```python
from build123d import *

# Parameters (mm, degrees)
SKETCH_1_R          = 21
SKETCH_1_R_2        = 7.5
EXTRUDE_1_DEPTH     = 13
EXTRUDE_2_DEPTH     = 6.5
FILLET_1_R          = 4
FILLET_2_R          = 2
SKETCH_3_R          = 3.5
CUT_EXTRUDE_1_DEPTH = 6.5
SKETCH_4_R          = 18
CUT_EXTRUDE_2_DEPTH = 2


with BuildPart() as part:
    # 草图1 → 凸台-拉伸1 (new body)
    with BuildSketch(Plane(origin=(0, 0, 0), x_dir=(1, 0, 0), z_dir=(0, 1, 0))):
        with Locations(Location((0, 0, 0), (0, 0, 90))):
            Circle(SKETCH_1_R)
        with Locations(Location((0, 0, 0), (0, 0, 90))):
            Circle(SKETCH_1_R_2, mode=Mode.SUBTRACT)
    extrude(amount=EXTRUDE_1_DEPTH)

    # 草图2 → 凸台-拉伸2 (add)
    with BuildSketch(Plane.XZ):
        with BuildLine():
            Line((32.727876998, 4.229192264), (19.975971523, 6.477697255))
            ThreePointArc((19.975971523, 6.477697255), (21, 0), (19.975971523, -6.477697255))
            Line((19.975971523, -6.477697255), (32.727876998, -4.229192264))
            ThreePointArc((32.727876998, -4.229192264), (33, 0), (32.727876998, 4.229192264))
        make_face()
        with BuildLine():
            Line((-32.727876998, -4.229192264), (-19.975971523, -6.477697255))
            ThreePointArc((-19.975971523, -6.477697255), (-21, 0), (-19.975971523, 6.477697255))
            Line((-19.975971523, 6.477697255), (-32.727876998, 4.229192264))
            ThreePointArc((-32.727876998, 4.229192264), (-33, 0), (-32.727876998, -4.229192264))
        make_face()
    extrude(amount=-EXTRUDE_2_DEPTH)

    # 圆角1
    fillet_1_edges = [part.edges().sort_by_distance(p)[0] for p in [
        (19.975971523, 3.25, -6.477697255),
        (19.975971523, 3.25, 6.477697255),
        (-19.975971523, 3.25, 6.477697255),
        (-19.975971523, 3.25, -6.477697255),
    ]]
    fillet(fillet_1_edges, radius=FILLET_1_R)

    # 圆角2
    fillet_2_edges = [part.edges().sort_by_distance(p)[0] for p in [
        (32.727876998, 3.25, 4.229192264),
        (32.727876998, 3.25, -4.229192264),
        (-32.727876998, 3.25, -4.229192264),
        (-32.727876998, 3.25, 4.229192264),
    ]]
    fillet(fillet_2_edges, radius=FILLET_2_R)

    # 草图3 → 切除-拉伸1 (cut)
    with BuildSketch(Plane(origin=(0, 6.5, 0), x_dir=(1, 0, 0), z_dir=(0, 1, 0))):
        with Locations(Location((-26.5, 0, 0), (0, 0, 270))):
            Circle(SKETCH_3_R)
        with Locations(Location((26.5, 0, 0), (0, 0, 270))):
            Circle(SKETCH_3_R)
    extrude(amount=-CUT_EXTRUDE_1_DEPTH, mode=Mode.SUBTRACT)

    # 草图4 → 切除-拉伸2 (cut)
    with BuildSketch(Plane.XZ):
        with Locations(Location((0, 0, 0), (0, 0, 270))):
            Circle(SKETCH_4_R)
    extrude(amount=-CUT_EXTRUDE_2_DEPTH, mode=Mode.SUBTRACT)


solid = part.part
```
Check sheet for the modelled part. Datum: model origin and axes. Units: mm. Give positions to 0.01 mm unless a question says otherwise; leave off trailing zeros. Loops run counter-clockwise (first coordinate to the right, second up) from the corner with the lowest first, then second, coordinate; pieces in that order, holes last. Notation, with made-up numbers: M 49,-24 L 61,-24 A5 cw 61,-17 Z; hole C 57.5,-14 d4. An arc over 180 degrees is marked long. Answer as CSV lines item,"result".
Item 1: Sectioned sample at D-D, the plane z = -10.5. Enter the section's corners in (x, y).
Reply:
outline,"M -18.19,0 L -14.62,0 L -14.62,2 L 14.62,2 L 14.62,0 L 18.19,0 L 18.19,13 L -18.19,13 Z"
Item 2: Sectioned sample at A-A, the plane x = 0. Enter the section's corners in (y, z), then the cut area to 3 significant figures.
Reply:
outline,"M 0,-21 L 13,-21 L 13,-7.5 L 2,-7.5 L 2,-18 L 0,-18 Z; M 0,18 L 2,18 L 2,7.5 L 13,7.5 L 13,21 L 0,21 Z"
area,"309 mm^2"
Item 3: Draft check along Z on faces 1 (the face through (-0.33, 7.423, 7.493)), 2 (the face through (-20.408, 3.296, -6.896)), 3 (the face through (-33, 3, 0)), 4 (the face through (-15, 0, -11)). Enter one of: pulls with the +Z half, pulls with the -Z half, needs draft (parallel to the pull), parting line crosses it, or undercut.
Reply:
face 1,"undercut"
face 2,"pulls with the -Z half"
face 3,"parting line crosses it"
face 4,"needs draft"
Item 4: Depth check by flat-ended pin: pin 1 Ø1.5 at (x, y) = (13, 10) entering from -Z; pin 2 Ø2 at (x, y) = (-22, 6.5) entering from -Z; pin 3 Ø4 at (x, y) = (-2.5, 8.5) entering from -Z; pin 4 Ø5.5 at (x, z) = (26.5, 0) entering from -Y. Enter the tip coordinate at first touch or a pass-through.
Reply:
pin 1,"z = -17.06"
pin 2,"z = -6.5"
pin 3,"z = -20.99"
pin 4,"through"
Item 5: Sectioned sample at B-B, the plane z = 0. Enter the section's corners in (x, y), then the cut area to 3 significant figures.
Reply:
outline,"M -33,0 L -30,0 L -30,6.5 L -33,6.5 Z; M -23,0 L -18,0 L -18,2 L -7.5,2 L -7.5,13 L -21,13 L -21,6.5 L -23,6.5 Z; M 7.5,2 L 18,2 L 18,0 L 23,0 L 23,6.5 L 21,6.5 L 21,13 L 7.5,13 Z; M 30,0 L 33,0 L 33,6.5 L 30,6.5 Z"
area,"374 mm^2"
Item 6: Scan lines: L1, parallel to X at y = 10.25, z = 0; L2, parallel to Y at x = -11.5, z = -12; L3, parallel to Z at x = -6, y = 5.75. Record each from-to range of solid material in increasing order.
Reply:
L1,"-21 to -7.5, 7.5 to 21"
L2,"2 to 13"
L3,"-20.12 to -4.5, 4.5 to 20.12"
Item 7: Sectioned sample at C-C, the plane y = 9.5. Enter the section's corners in (x, z).
Reply:
outline,"C 0,0 d42; hole C 0,0 d15"
